```python
from build123d import *

# Parameters (mm, degrees)
SKETCH1_W           = 70
SKETCH1_H           = 83
BOSS_EXTRUDE1_DEPTH = 6
SKETCH2_W           = 70
SKETCH2_H           = 8
BOSS_EXTRUDE2_DEPTH = 30
SKETCH3_R           = 20
CUT_EXTRUDE1_DEPTH  = 20
SKETCH4_W           = 20
SKETCH4_H           = 12.019208042
CUT_EXTRUDE2_DEPTH  = 20
SKETCH5_R           = 1.25
CUT_EXTRUDE3_DEPTH  = 20
CUT_EXTRUDE4_DEPTH  = 20
SKETCH7_W           = 0.5
SKETCH7_H           = 25
CUT_EXTRUDE5_DEPTH  = 90
FILLET1_R           = 2
CHAMFER1_SIZE       = 2


with BuildPart() as part:
    # Sketch1 → Boss-Extrude1 (new body)
    with BuildSketch(Plane(origin=(0, 0, 0), x_dir=(1, 0, 0), z_dir=(0, 1, 0))):
        Rectangle(SKETCH1_W, SKETCH1_H)
    extrude(amount=BOSS_EXTRUDE1_DEPTH)

    # Sketch2 → Boss-Extrude2 (add)
    with BuildSketch(Plane(origin=(0, 6, 0), x_dir=(1, 0, 0), z_dir=(0, 1, 0))):
        with Locations((0, -37.5)):
            Rectangle(SKETCH2_W, SKETCH2_H)
    extrude(amount=BOSS_EXTRUDE2_DEPTH)

    # Sketch3 → Cut-Extrude1 (cut)
    with BuildSketch(Plane.XZ):
        with Locations(Location((0, -8.5, 0), (0, 0, 270))):
            Circle(SKETCH3_R)
    extrude(amount=-CUT_EXTRUDE1_DEPTH, mode=Mode.SUBTRACT)

    # Sketch4 → Cut-Extrude2 (cut)
    with BuildSketch(Plane(origin=(0, 6, 0), x_dir=(1, 0, 0), z_dir=(0, 1, 0))):
        with Locations((0, 41.509604021)):
            Rectangle(SKETCH4_W, SKETCH4_H)
    extrude(amount=-CUT_EXTRUDE2_DEPTH, mode=Mode.SUBTRACT)

    # Sketch5 → Cut-Extrude3 (cut)
    with BuildSketch(Plane(origin=(0, 6, 0), x_dir=(1, 0, 0), z_dir=(0, 1, 0))):
        with Locations(Location((31, 8.5, 0), (0, 0, 270))):
            Circle(SKETCH5_R)
        with Locations(Location((15.5, -18.346787517, 0), (0, 0, 270))):
            Circle(SKETCH5_R)
        with Locations(Location((-15.5, -18.346787517, 0), (0, 0, 270))):
            Circle(SKETCH5_R)
        with Locations(Location((-31, 8.5, 0), (0, 0, 270))):
            Circle(SKETCH5_R)
        with Locations(Location((-15.5, 35.346787517, 0), (0, 0, 270))):
            Circle(SKETCH5_R)
        with Locations(Location((15.5, 35.346787517, 0), (0, 0, 270))):
            Circle(SKETCH5_R)
    extrude(amount=-CUT_EXTRUDE3_DEPTH, mode=Mode.SUBTRACT)

    # Sketch6 → Cut-Extrude4 (cut)
    with BuildSketch(Plane(origin=(0, 0, 33.5), x_dir=(-1, 0, 0), z_dir=(0, 0, -1))):
        with BuildLine():
            Line((25, 17.8), (-25, 17.8))
            ThreePointArc((-25, 17.8), (-28.2, 21), (-25, 24.2))
            Line((-25, 24.2), (25, 24.2))
            ThreePointArc((25, 24.2), (28.2, 21), (25, 17.8))
        make_face()
    extrude(amount=-CUT_EXTRUDE4_DEPTH, mode=Mode.SUBTRACT)

    # Sketch7 → Cut-Extrude5 (cut)
    with BuildSketch(Plane.ZY.offset(35)):
        with Locations((41.25, 18.5)):
            Rectangle(SKETCH7_W, SKETCH7_H)
    extrude(amount=-CUT_EXTRUDE5_DEPTH, mode=Mode.SUBTRACT)

    # Fillet1
    fillet1_edges = [part.edges().sort_by_distance(p)[0] for p in [
        (-10, 3, -35.5),
        (10, 3, -35.5),
    ]]
    fillet(fillet1_edges, radius=FILLET1_R)

    # Chamfer1
    chamfer1_edges = [part.edges().sort_by_distance(p)[0] for p in [
        (-35, 36, 37.5),
        (35, 36, 37.5),
        (-10, 3, -41.5),
        (10, 3, -41.5),
        (-35, 3, -41.5),
        (35, 3, -41.5),
    ]]
    chamfer(chamfer1_edges, length=CHAMFER1_SIZE)


solid = part.part
```
Part model, mm, in its own coordinate system. A direction names the side the tool comes from. Coordinates: 2 decimals unless noted, no trailing zeros. Write each loop counter-clockwise with the first axis right and the second up, starting at its lowest first coordinate (ties: lowest second). Pieces come first, ordered by that corner, then holes.
Item 1: Slice it at B-B (x = -23). Write the cut outline in (y, z).
Item 2: Slice it at D-D (x = 0). Write the cut outline in (y, z), and give its area (4 significant figures).
Item 3: Mould opens along X. For faces 5 (the face through (0, 6, 12)), 6 (the face through (11, 3, -40.5)), 7 (the face through (35, 4, 13)) say: released by +X, released by -X, zero draft, split by the parting line, or undercut.
Item 4: Pin check, flat tips, straight feed: pin 1 (2 mm diameter, centred on x = -31, z = -8.5, fed in from +Y); pin 2 (10 mm diameter, centred on x = 26, y = 22, fed in from +Z); pin 3 (3 mm diameter, centred on x = -19, y = 23, fed in from -Z); pin 4 (6.5 mm diameter, centred on x = -2.5, y = 1.5, fed in from -Z). Stop position of each tip, or through.
Item 5: Slice it at A-A (z = -8.5). Write the cut outline in (x, y).
Item 6: Which spindle directions (+Z, -Z, +X, -X, +Y, -Y) get a long thin tool onto all of the face, cutting with end or side? Do faces 1 (the face through (-10, 3, -38)), 2 (the face through (0, 17, 33.5)), 3 (the face through (22, 3, -41.5)), 4 (the face through (0, 24.2, 37)). Say none if no direction does.
Item 7: Slice it at C-C (y = 21). Write the cut outline in (x, z), and give its area (3 significant figures).
Item 8: Probe line 1 (X direction, y = 2, z = 17.5); line 2 (Z direction, x = 15, y = 3); line 3 (Z direction, x = -18, y = 12). List the from-to ranges inside material, lowest first.
Results found:
1. outline: (0, -41.5) - (6, -41.5) - (6, 33.5) - (17.8, 33.5) - (17.8, 41) - (6, 41) - (6, 41.5) - (0, 41.5) - close; (24.2, 33.5) - (36, 33.5) - (36, 41.5) - (31, 41.5) - (31, 41) - (24.2, 41) - close
2. outline: (0, -35.5) - (6, -35.5) - (6, -28.5) - (0, -28.5) - close; (0, 11.5) - (6, 11.5) - (6, 33.5) - (17.8, 33.5) - (17.8, 41) - (6, 41) - (6, 41.5) - (0, 41.5) - close; (24.2, 33.5) - (36, 33.5) - (36, 41.5) - (31, 41.5) - (31, 41) - (24.2, 41) - close
2. area: 401.5 mm2
3. face 5: zero draft
3. face 6: undercut
3. face 7: released by +X
4. pin 1: passes through
4. pin 2: stops at z = 41
4. pin 3: stops at z = 33.5
4. pin 4: stops at z = -35.5
5. outline: (-35, 0) - (-32.25, 0) - (-32.25, 6) - (-35, 6) - close; (-29.75, 0) - (-20, 0) - (-20, 6) - (-29.75, 6) - close; (20, 0) - (29.75, 0) - (29.75, 6) - (20, 6) - close; (32.25, 0) - (35, 0) - (35, 6) - (32.25, 6) - close
6. face 1: -Z, +Y, -Y
6. face 2: -Z, +X, -X, +Y
6. face 3: -Z, +X, -X, +Y, -Y
6. face 4: +Z, -Z
7. outline: (-35, 33.5) - (-28.2, 33.5) - (-28.2, 41) - (-35, 41) - close; (28.2, 33.5) - (35, 33.5) - (35, 41) - (28.2, 41) - close
7. area: 102 mm2
8. line 1: x = -35 to -16.42, -14.58 to 14.58, 16.42 to 35
8. line 2: z = -41.5 to -36.49, -34.2 to -21.73, 4.73 to 17.2, 19.49 to 41.5
8. line 3: z = 33.5 to 41
